from build123d import *

# Parameters (mm, degrees)
SKETCH_1_W                   = 92
SKETCH_1_H                   = 60
EXTRUDE_1_DEPTH              = 144
HOLE_WIZARD_M4_1_D           = 4.5
HOLE_WIZARD_M4_1_CBORE_D     = 8
HOLE_WIZARD_M4_1_CBORE_DEPTH = 35
CHAMFER_1_SIZE               = 2
HOLE_WIZARD_M4_2_D           = 4.5
HOLE_WIZARD_M4_2_CBORE_D     = 8
HOLE_WIZARD_M4_2_CBORE_DEPTH = 37


with BuildPart() as part:
    # 草图1 → 凸台-拉伸1 (new body)
    with BuildSketch(Plane.XY):
        Rectangle(SKETCH_1_W, SKETCH_1_H)
    extrude(amount=EXTRUDE_1_DEPTH)

    # M4 六角凹头螺钉的柱形沉头孔1 (through all)
    with Locations(Plane.XY.offset(144)):
        with Locations((-41, 20), (-41, -20), (41, 20), (41, -20)):
            CounterBoreHole(HOLE_WIZARD_M4_1_D / 2, HOLE_WIZARD_M4_1_CBORE_D / 2, HOLE_WIZARD_M4_1_CBORE_DEPTH)

    # 倒角1
    chamfer_1_edges = [part.edges().sort_by_distance(p)[0] for p in [
        (46, -30, 72),
        (-46, -30, 72),
        (-46, 30, 72),
        (46, 30, 72),
    ]]
    chamfer(chamfer_1_edges, length=CHAMFER_1_SIZE)

    # M4 六角凹头螺钉的柱形沉头孔2 (through all)
    with Locations(Plane(origin=(0, 0, 0), x_dir=(-1, 0, 0), z_dir=(0, 0, -1))):
        with Locations((0, 17.7), (-27, -19.9), (27, -19.9)):
            CounterBoreHole(HOLE_WIZARD_M4_2_D / 2, HOLE_WIZARD_M4_2_CBORE_D / 2, HOLE_WIZARD_M4_2_CBORE_DEPTH)


solid = part.part
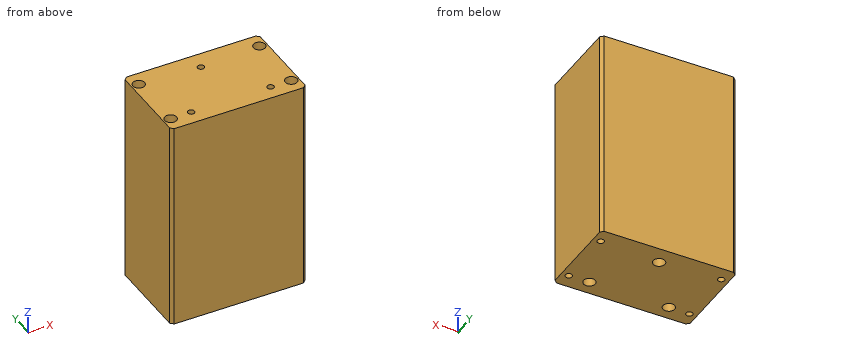
Source: CAD feature listing. Evaluate the final solid. Frame: model axes, mm. Coordinates: 2 decimals unless noted, no trailing zeros. Loops run counter-clockwise (first coordinate to the right, second up) from the corner with the lowest first, then second, coordinate; pieces in that order, holes last. Notation, with made-up numbers: (-19.5, 51.25) -> (37.5, 51.25) arc R13 ccw to (37.5, 59.25) -> close; hole circle Ø4 at (13, -31). An arc over 180 degrees is marked (long way). Answer in a Markdown table with one row per item. Add a question column.
Q1. Section D-D on z = 123. Return the cut outline in (x, y), and give its area (3 significant figures).
Q2. Contact query for flat-ended pins moving along their axis: pin 1 Ø5 at (x, y) = (-27, -19.9) entering from -Z; pin 2 Ø4 at (x, y) = (-40, -19) entering from +Z. Output: stop coordinate, or through.
Q3. Section A-A on x = 27. Return the cut outline in (y, z), and give its area (3 significant figures).
Q4. Section C-C on x = -41. Return the cut outline in (y, z).
Q5. Section B-B on z = 40.5. Return the cut outline in (x, y), and give its area (3 significant figures).
Q6. Ray query, line 1 along Y through (x, z) = (41, 65); line 2 along Y through (x, z) = (41, 130.5); line 3 along X through (y, z) = (-19, 69). Return the intervals inside material, ascending.
Computed values:
| question | item | result |
|---|---|---|
| 1 | outline | (-46, -28) -> (-44, -30) -> (44, -30) -> (46, -28) -> (46, 28) -> (44, 30) -> (-44, 30) -> (-46, 28) -> close; hole circle Ø8 at (-41, -20); hole circle Ø8 at (-41, 20); hole circle Ø4.5 at (-27, -19.9); hole circle Ø4.5 at (0, 17.7); hole circle Ø4.5 at (27, -19.9); hole circle Ø8 at (41, -20); hole circle Ø8 at (41, 20) |
| 1 | area | 5,260 mm^2 |
| 2 | pin 1 | stops at z = 37 |
| 2 | pin 2 | stops at z = 109 |
| 3 | outline | (-30, 0) -> (-23.9, 0) -> (-23.9, 37) -> (-22.15, 37) -> (-22.15, 144) -> (-30, 144) -> close; (-17.65, 37) -> (-15.9, 37) -> (-15.9, 0) -> (30, 0) -> (30, 144) -> (-17.65, 144) -> close |
| 3 | area | 7,860 mm^2 |
| 4 | outline | (-30, 0) -> (-22.25, 0) -> (-22.25, 109) -> (-24, 109) -> (-24, 144) -> (-30, 144) -> close; (-17.75, 0) -> (17.75, 0) -> (17.75, 109) -> (16, 109) -> (16, 144) -> (-16, 144) -> (-16, 109) -> (-17.75, 109) -> close; (22.25, 0) -> (30, 0) -> (30, 144) -> (24, 144) -> (24, 109) -> (22.25, 109) -> close |
| 5 | outline | (-46, -28) -> (-44, -30) -> (44, -30) -> (46, -28) -> (46, 28) -> (44, 30) -> (-44, 30) -> (-46, 28) -> close; hole circle Ø4.5 at (-41, -20); hole circle Ø4.5 at (-41, 20); hole circle Ø4.5 at (-27, -19.9); hole circle Ø4.5 at (0, 17.7); hole circle Ø4.5 at (27, -19.9); hole circle Ø4.5 at (41, -20); hole circle Ø4.5 at (41, 20) |
| 5 | area | 5,400 mm^2 |
| 6 | line 1 | y = -30 to -22.25, -17.75 to 17.75, 22.25 to 30 |
| 6 | line 2 | y = -30 to -24, -16 to 16, 24 to 30 |
| 6 | line 3 | x = -46 to -43.02, -38.98 to -29.06, -24.94 to 24.94, 29.06 to 38.98, 43.02 to 46 |
